Could you check a few things on this drawing? It's one solid part, dimensions in mm from its lowest x, y, z. Coordinates: 2 decimals unless noted, no trailing zeros. Loops run counter-clockwise (first coordinate to the right, second up) from the corner with the lowest first, then second, coordinate; pieces in that order, holes last. Notation, with made-up numbers: M 81.25,45.5 L 96.25,45.5 A16 ccw 96.25,49.5 Z; hole C -24.75,79 d2. An arc over 180 degrees is marked long. Use one line per item in the form item = value. Start each with the question number.
(1) Will these pins go through, and if not, where does the flat tip stop? P1, Ø3, axis at x = 1.5, z = 4.5, coming from the -Y side; P2, Ø2, axis at x = 9.5, z = 2, coming from the -Y side (1 decimal); P3, Ø4, axis at x = 11, z = 4, coming from the -Y side.
(2) Please list where these lines run through material, in increasing order: L1, parallel to X at y = 7.5, z = 5.5; L2, parallel to X at y = 8.5, z = 6 (1 decimal); L3, parallel to Y at x = 7.5, z = 4.5 (1 decimal).
(3) Thinking about a two-plate mould opening in Y: for the marked faces 1, 2 and 3, which applies, +Y half, -Y half, draft (parallel to the pull), parting line (faces both ways), or undercut?
(4) Imagine slicing it at A-A, the plane z = 6. Please give me the cut outline in (x, y) (1 decimal).
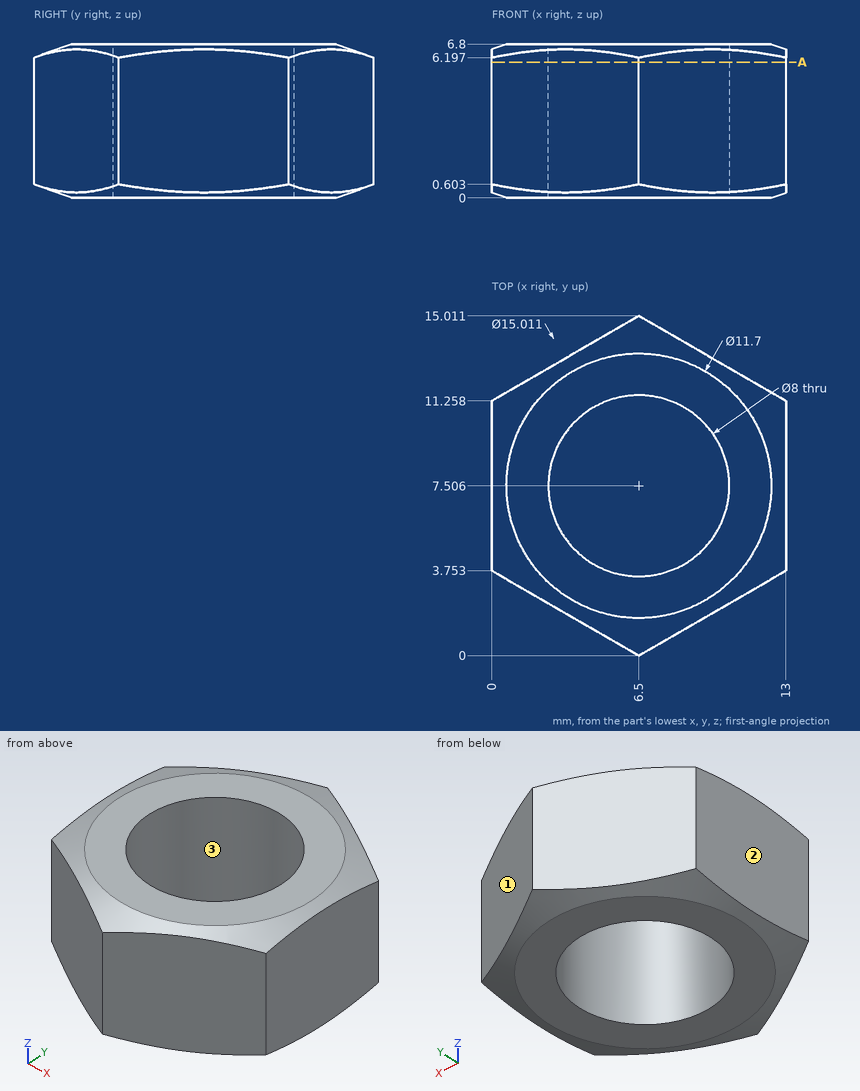
Answer:
q1.P1 = 2.02
q1.P2 = 1.2
q1.P3 = 1.44
q2.L1 = 0 to 2.5, 10.5 to 13
q2.L2 = 0 to 2.6, 10.4 to 13
q2.L3 = 0.6 to 3.6, 11.4 to 14.4
q3.face_1 = +Y half
q3.face_2 = draft
q3.face_3 = undercut
q4.outline = M 0,3.8 L 6.5,0 L 13,3.8 L 13,11.3 L 6.5,15 L 0,11.3 Z; hole C 6.5,7.5 d8
